from build123d import *

# Parameters (mm, degrees)
SKETCH_1_W          = 215
SKETCH_1_H          = 115
EXTRUDE_1_DEPTH     = 30
SKETCH_2_R          = 2.5
CUT_EXTRUDE_1_DEPTH = 30


with BuildPart() as part:
    # 草图1 → 凸台-拉伸1 (new body)
    with BuildSketch(Plane(origin=(0, 0, 0), x_dir=(1, 0, 0), z_dir=(0, 1, 0))):
        Rectangle(SKETCH_1_W, SKETCH_1_H)
    extrude(amount=EXTRUDE_1_DEPTH)

    # 草图2 → 切除-拉伸1 (cut)
    with BuildSketch(Plane(origin=(0, 30, 0), x_dir=(1, 0, 0), z_dir=(0, 1, 0))):
        with Locations(Location((-75, 25, 0), (0, 0, 270))):
            Circle(SKETCH_2_R)
        with Locations(Location((75, 25, 0), (0, 0, 270))):
            Circle(SKETCH_2_R)
        with Locations(Location((75, -25, 0), (0, 0, 270))):
            Circle(SKETCH_2_R)
        with Locations(Location((-75, -25, 0), (0, 0, 270))):
            Circle(SKETCH_2_R)
    extrude(amount=-CUT_EXTRUDE_1_DEPTH, mode=Mode.SUBTRACT)


solid = part.part
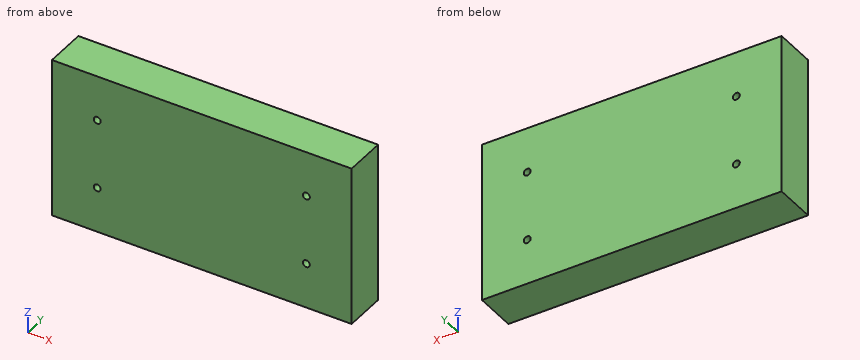
Work out the finished part from the listing and answer in its coordinate system (mm). Round coordinates to 2 decimals unless told otherwise and drop trailing zeros. Write each loop counter-clockwise with the first axis right and the second up, starting at its lowest first coordinate (ties: lowest second). Pieces come first, ordered by that corner, then holes.
1) Straight lines are drawn through the part: line 1 (X direction, y = 10.5, z = 25); line 2 (X direction, y = 19.5, z = 27). For each, find the intervals that lie inside material, in ascending order.
2) A cutting plane is placed at A-A (x = -75). Give the vertices of the cut face in (y, z), plus the area to 3 significant figures.
3) A cutting plane is placed at B-B (z = 25). Give the vertices of the cut face in (x, y).
Completed:
1. line 1: x = -107.5 to -77.5, -72.5 to 72.5, 77.5 to 107.5
1. line 2: x = -107.5 to -76.5, -73.5 to 73.5, 76.5 to 107.5
2. outline: (0, -57.5) - (30, -57.5) - (30, -27.5) - (0, -27.5) - close; (0, -22.5) - (30, -22.5) - (30, 22.5) - (0, 22.5) - close; (0, 27.5) - (30, 27.5) - (30, 57.5) - (0, 57.5) - close
2. area: 3,150 mm2
3. outline: (-107.5, 0) - (-77.5, 0) - (-77.5, 30) - (-107.5, 30) - close; (-72.5, 0) - (72.5, 0) - (72.5, 30) - (-72.5, 30) - close; (77.5, 0) - (107.5, 0) - (107.5, 30) - (77.5, 30) - close
